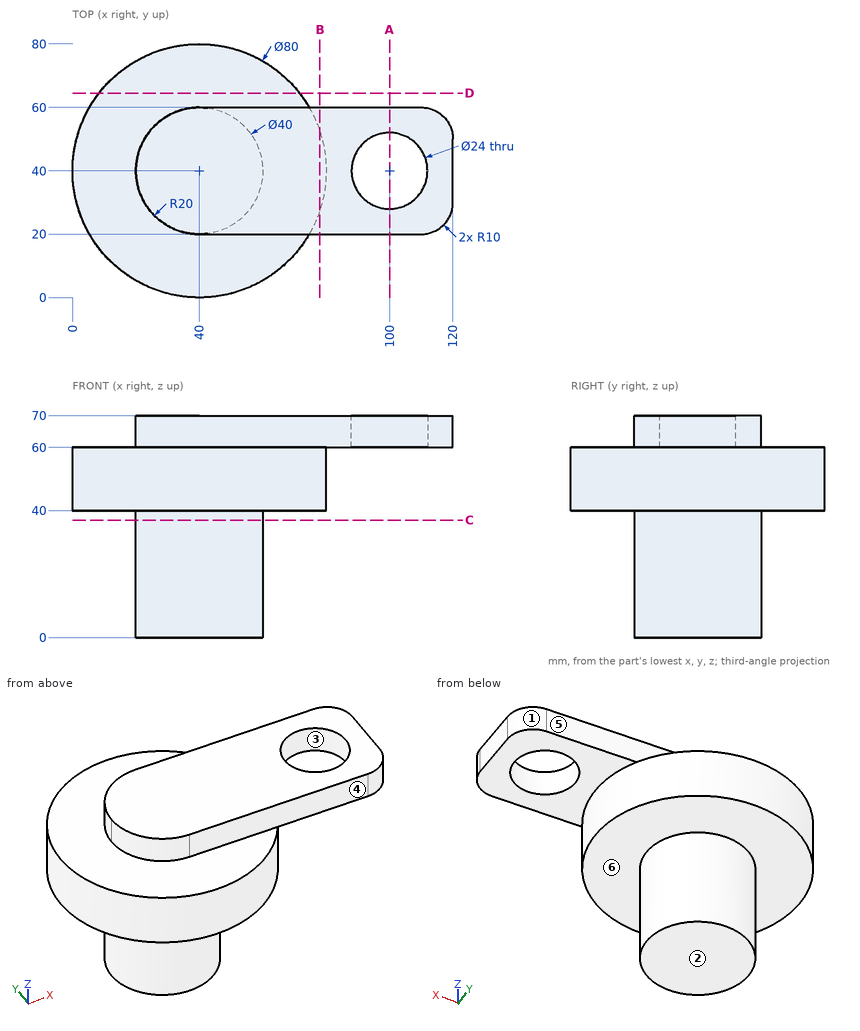
Drawing for the job (mm, zero at the part's lowest x, y, z). A direction names the side the tool comes from. Round coordinates to 2 decimals unless told otherwise and drop trailing zeros. Order: outer loops, then holes, each group sorted by start corner. A loop starts at its lowest first (then second) coordinate and runs counter-clockwise, first axis right, second up.
Item 1: Mould opens along Y. For the marked faces 1, 2 and 3 say: pulls with the +Y half, pulls with the -Y half, needs draft (parallel to the pull), parting line crosses it, or undercut.
Item 2: Probe line 1 along Y through (x, z) = (100, 65.25); line 2 along Z through (x, y) = (60, 14); line 3 along Z through (x, y) = (61.5, 24). List the from-to ranges inside material, lowest first.
Item 3: Saw through at C-C on z = 37. Write the cut outline in (x, y), then the cut area to 3 significant figures.
Item 4: Saw through at B-B on x = 78. Write the cut outline in (y, z).
Item 5: Saw through at D-D on y = 64.5. Write the cut outline in (x, z).
Item 6: Pin check, flat tips, straight feed: pin 1 (1.5 mm diameter, centred on x = 101, y = 51.5, fed in from -Z); pin 2 (3 mm diameter, centred on x = 46.5, z = 20, fed in from +Y); pin 3 (8 mm diameter, centred on x = 77.5, z = 64.5, fed in from +Y); pin 4 (12 mm diameter, centred on x = 101.5, y = 45, fed in from -Z). Stop position of each tip, or through.
Item 7: Saw through at A-A on x = 100. Write the cut outline in (y, z).
Item 8: Tool access for the marked faces 4, 5 and 6: list every direction of +Z, -Z, +X, -X, +Y, -Y with a clear straight run to the whole face (end or side of a thin tool).
Reported:
1. face 1: pulls with the +Y half
1. face 2: needs draft
1. face 3: undercut
2. line 1: y = 20 to 28, 52 to 60
2. line 2: z = 40 to 60
2. line 3: z = 40 to 70
3. outline: circle Ø40 at (40, 40)
3. area: 1,260 mm2
4. outline: (20, 60) - (27.51, 60) - (27.51, 40) - (52.49, 40) - (52.49, 60) - (60, 60) - (60, 70) - (20, 70) - close
5. outline: (8.38, 40) - (71.62, 40) - (71.62, 60) - (8.38, 60) - close
6. pin 1: stops at z = 60
6. pin 2: stops at y = 59.36
6. pin 3: stops at y = 60
6. pin 4: passes through
7. outline: (20, 60) - (28, 60) - (28, 70) - (20, 70) - close; (52, 60) - (60, 60) - (60, 70) - (52, 70) - close
8. face 4: +Z, +X, -X, -Y
8. face 5: +Z, +X, -X, +Y
8. face 6: -Z
